The model under review builds one solid part; all positions refer to its coordinate system, in mm. Coordinates: 2 decimals unless noted, no trailing zeros. Loops run counter-clockwise (first coordinate to the right, second up) from the corner with the lowest first, then second, coordinate; pieces in that order, holes last. Notation, with made-up numbers: (47.25, 71) - (76.25, 71) arc R22 cw to (76.25, 85) - close; hole circle Ø4 at (-16, -30). An arc over 180 degrees is marked (long way). Use a Markdown table: item, result. Add a question column.
1) Add section C-C, the plane z = 2.25. Give the boundary of the cut face in (x, y), and give its area (3 significant figures).
2) Add section A-A, the plane y = 0. Give the boundary of the cut face in (x, z).
3) The part is to be moulded in two halves that separate along Y. For faces 1 (the flat face through (0, 37.5, 3)), 2 (the flat face through (0, -37.5, 3)), 3 (the cylindrical face through (0, -19, 3)), say which applies: pulls with the +Y half, pulls with the -Y half, needs draft (parallel to the pull), parting line crosses it, or undercut.
4) Add section B-B, the plane x = -2.25. Give the boundary of the cut face in (y, z).
5) To check wall thickness, follow L1, parallel to Y at x = 0, z = 3; L2, parallel to Y at x = 1.5, z = 5; L3, parallel to X at y = 23, z = 5. State the ranges of each line that lie inside material, in increasing order. Write a range as [from, to].
6) Clearance check with a flat-ended pin moving along its axis: pin 1 (4 mm diameter, centred on x = 0, y = -22.5, fed in from +Z). State where the tip first meets the part, or that it passes through.
```python
from build123d import *

# Parameters (mm, degrees)
SKETCH_1_W            = 30
SKETCH_1_H            = 75
EXTRUDE_1_DEPTH       = 6.5
HOLE_WIZARD_7_0_7_1_D = 7
CHAMFER_1_SIZE        = 1


with BuildPart() as part:
    # 草图1 → 凸台-拉伸1 (new body)
    with BuildSketch(Plane.XY):
        Rectangle(SKETCH_1_W, SKETCH_1_H)
    extrude(amount=EXTRUDE_1_DEPTH)

    # Ø7.0 (7) 直径孔1 (through all)
    with Locations(Plane.XY.offset(6.5)):
        with Locations((0, 0), (0, -22.5), (0, 22.5)):
            Hole(HOLE_WIZARD_7_0_7_1_D / 2)

    # 倒角1
    chamfer_1_edges = [part.edges().sort_by_distance(p)[0] for p in [
        (15, -37.5, 3.25),
        (-15, -37.5, 3.25),
        (-15, 37.5, 3.25),
        (15, 37.5, 3.25),
    ]]
    chamfer(chamfer_1_edges, length=CHAMFER_1_SIZE)


solid = part.part
```
From the geometry:
| question | item | result |
|---|---|---|
| 1 | outline | (-15, -36.5) - (-14, -37.5) - (14, -37.5) - (15, -36.5) - (15, 36.5) - (14, 37.5) - (-14, 37.5) - (-15, 36.5) - close; hole circle Ø7 at (0, -22.5); hole circle Ø7 at (0, 0); hole circle Ø7 at (0, 22.5) |
| 1 | area | 2,130 mm^2 |
| 2 | outline | (-15, 0) - (-3.5, 0) - (-3.5, 6.5) - (-15, 6.5) - close; (3.5, 0) - (15, 0) - (15, 6.5) - (3.5, 6.5) - close |
| 3 | face 1 | pulls with the +Y half |
| 3 | face 2 | pulls with the -Y half |
| 3 | face 3 | undercut |
| 4 | outline | (-37.5, 0) - (-25.18, 0) - (-25.18, 6.5) - (-37.5, 6.5) - close; (-19.82, 0) - (-2.68, 0) - (-2.68, 6.5) - (-19.82, 6.5) - close; (2.68, 0) - (19.82, 0) - (19.82, 6.5) - (2.68, 6.5) - close; (25.18, 0) - (37.5, 0) - (37.5, 6.5) - (25.18, 6.5) - close |
| 5 | L1 | y = [-37.5, -26], [-19, -3.5], [3.5, 19], [26, 37.5] |
| 5 | L2 | y = [-37.5, -25.66], [-19.34, -3.16], [3.16, 19.34], [25.66, 37.5] |
| 5 | L3 | x = [-15, -3.46], [3.46, 15] |
| 6 | pin 1 | passes through |
